from build123d import *

# Parameters (mm, degrees)
KEY_BODY_DEPTH         = 20
SHANK_SLOT_SKETCH_W    = 10
SHANK_SLOT_SKETCH_H    = 35
SHANK_SLOT_DEPTH       = 20
GRIP_HOLES_SKETCH_R    = 10
GRIP_HOLES_2X_20_DEPTH = 20


with BuildPart() as part:
    # Key Profile Sketch → Key Body (new body)
    with BuildSketch(Plane.XY):
        with BuildLine():
            Line((25, -87), (30, -87))
            Line((30, -87), (30, -42))
            Line((30, -42), (35, -42))
            ThreePointArc((35, -42), (38.629636909, -27.380389945), (50, -17.5))
            ThreePointArc((50, -17.5), (67.350600333, 2.28181246), (45.475335312, 16.904952217))
            ThreePointArc((45.475335312, 16.904952217), (23.461156875, 14.723275331), (1.505978003, 17.435080449))
            ThreePointArc((1.505978003, 17.435080449), (-17.483762579, 0.753688313), (0, -17.5))
            ThreePointArc((0, -17.5), (11.370363091, -27.380389945), (15, -42))
            Line((15, -42), (20, -42))
            Line((20, -42), (20, -87))
            Line((20, -87), (25, -87))
        make_face()
    extrude(amount=KEY_BODY_DEPTH)

    # Shank Slot Sketch → Shank Slot (cut)
    with BuildSketch(Plane(origin=(30, 0, 0), x_dir=(0, 0, -1), z_dir=(1, 0, 0))):
        with Locations((-10, -69.5)):
            Rectangle(SHANK_SLOT_SKETCH_W, SHANK_SLOT_SKETCH_H)
    extrude(amount=-SHANK_SLOT_DEPTH, mode=Mode.SUBTRACT)

    # Grip Holes Sketch → Grip Holes 2xØ20 (cut)
    with BuildSketch(Plane.XY.offset(20)):
        Circle(GRIP_HOLES_SKETCH_R)
        with Locations((50, 0)):
            Circle(GRIP_HOLES_SKETCH_R)
    extrude(amount=-GRIP_HOLES_2X_20_DEPTH, mode=Mode.SUBTRACT)


solid = part.part
Design review of the part built by this model. Coordinates are the model's own, in mm. A direction names the side the tool comes from. Give positions to 0.01 mm unless a question says otherwise; leave off trailing zeros. Loops run counter-clockwise (first coordinate to the right, second up) from the corner with the lowest first, then second, coordinate; pieces in that order, holes last. Notation, with made-up numbers: (-1.5, -14.5) -> (10.5, -14.5) arc R11 ccw to (10.5, -9.5) -> close; hole circle Ø1 at (25, 54). An arc over 180 degrees is marked (long way). One line per question, with ' | ' between items. Start each with the question number.
(1) We need section D-D (z = 17.25). State the section outline as (x, y) points.
(2) We need section B-B (x = 7.5). State the section outline as (y, z) points, and give its area (3 significant figures).
(3) Draft analysis for pull direction Y (two halves, no side actions). For faces 1 (the face through (23.77, 14.72, 9.86)), 2 (the face through (-2.17, -9.76, 10.14)), 3 (the face through (24, -11, 20)), 4 (the face through (40, 0, 10)), state which applies: +Y half, -Y half, draft (parallel to the pull), parting line (faces both ways), or undercut.
(4) We need section C-C (y = -80). State the section outline as (x, z) points.
(5) For line 1 (Y direction, x = 50, z = 8); line 2 (X direction, y = 4, z = 8.75); line 3 (Y direction, x = 33, z = 11.5), list the stretches that pass through material, from the lowest coordinate up.
(6) For faces 5 (the face through (25, -70, 15)), 6 (the face through (25, -87, 2)), 7 (the face through (32, -42, 10)), 8 (the face through (20, -59, 3)), 9 (the face through (24, -11, 0)), list the 3-axis set-ups (+Z, -Z, +X, -X, +Y, -Y) from which the entire face can be reached by the end or side of a thin tool; tool diameter is ignored.
(7) Insertion check: P1, Ø4, axis at y = -28, z = 17, coming from the -X side; P2, Ø6, axis at y = -8.5, z = 16.5, coming from the -X side; P3, Ø1, axis at x = 9.5, z = 7.5, coming from the +Y side. Each pin has a flat end and moves straight along its axis. Give the tip position at first contact, or say it passes through.
(8) We need section A-A (y = 0). State the section outline as (x, z) points.
The answers:
1) outline: (0, -17.5) arc R25 cw to (15, -42) -> (20, -42) -> (20, -87) -> (30, -87) -> (30, -42) -> (35, -42) arc R25 cw to (50, -17.5) arc R17.5 ccw (long way) to (45.48, 16.9) arc R100 cw to (1.51, 17.44) arc R17.5 ccw (long way) to start; hole circle Ø20 at (0, 0); hole circle Ø20 at (50, 0)
2) outline: (-22.53, 0) -> (-6.61, 0) -> (-6.61, 20) -> (-22.53, 20) -> close; (6.61, 0) -> (16.2, 0) -> (16.2, 20) -> (6.61, 20) -> close | area: 510 mm^2
3) face 1: +Y half | face 2: undercut | face 3: draft | face 4: undercut
4) outline: (20, 0) -> (30, 0) -> (30, 5) -> (20, 5) -> close; (20, 15) -> (30, 15) -> (30, 20) -> (20, 20) -> close
5) line 1: y = -17.5 to -10, 10 to 17.5 | line 2: x = -17.04 to -9.17, 9.17 to 40.83, 59.17 to 67.04 | line 3: y = -42 to 15.06
6) face 5: +X, -X, -Y | face 6: +Z, -Z, +X, -X, -Y | face 7: +Z, -Z, +X, -Y | face 8: +Z, -Z, -X, -Y | face 9: -Z, +X, -X, +Y, -Y
7) P1: stops at x = 10.46 | P2: stops at x = -16.61 | P3: stops at y = 15.95
8) outline: (-17.5, 0) -> (-10, 0) -> (-10, 20) -> (-17.5, 20) -> close; (10, 0) -> (40, 0) -> (40, 20) -> (10, 20) -> close; (60, 0) -> (67.5, 0) -> (67.5, 20) -> (60, 20) -> close
